Drawing for the job (mm, zero at the part's lowest x, y, z). A direction names the side the tool comes from. Round coordinates to 2 decimals unless told otherwise and drop trailing zeros. Loops run counter-clockwise (first coordinate to the right, second up) from the corner with the lowest first, then second, coordinate; pieces in that order, holes last. Notation, with made-up numbers: (-22, -31.5) -> (11, -31.5) arc R28 cw to (11, -1.5) -> close; hole circle Ø8 at (66, 71.5). An arc over 180 degrees is marked (long way). Put each result on its own line as item: value. Start each with the question number.
Item 1: Cut at C-C, the plane z = 2.5. List the corners of the cut face in (x, y).
Item 2: Drill centre lines: probe 1 along Y at (x, z) = (6, 2.5); probe 2 along Y at (x, z) = (8, 3.75); probe 3 along X at (y, z) = (4.25, 2.75). Where is each one in solid material? Low to high. Write a range as [from, to].
Item 3: Flat gauge pins, fed straight in: pin 1 Ø1.5 at (x, z) = (6, 2.5) entering from +Y; pin 2 Ø3.5 at (x, y) = (6.5, 7.5) entering from +Z; pin 3 Ø2 at (y, z) = (3.5, 1.5) entering from -X. Where does each tip first touch, or does it go through?
Item 4: Cut at B-B, the plane y = 6. List the corners of the cut face in (x, z), plus the area to 3 significant figures.
Item 5: Pull direction Y, two halves, no side cores. Call the marked faces 3, 4 and 5: +Y half, -Y half, draft (parallel to the pull), parting line (faces both ways), or undercut.
Item 6: Cut at A-A, the plane x = 6. List the corners of the cut face in (y, z).
Item 7: Tool access for the marked faces 1 and 2: list every direction of +Z, -Z, +X, -X, +Y, -Y with a clear straight run to the whole face (end or side of a thin tool).
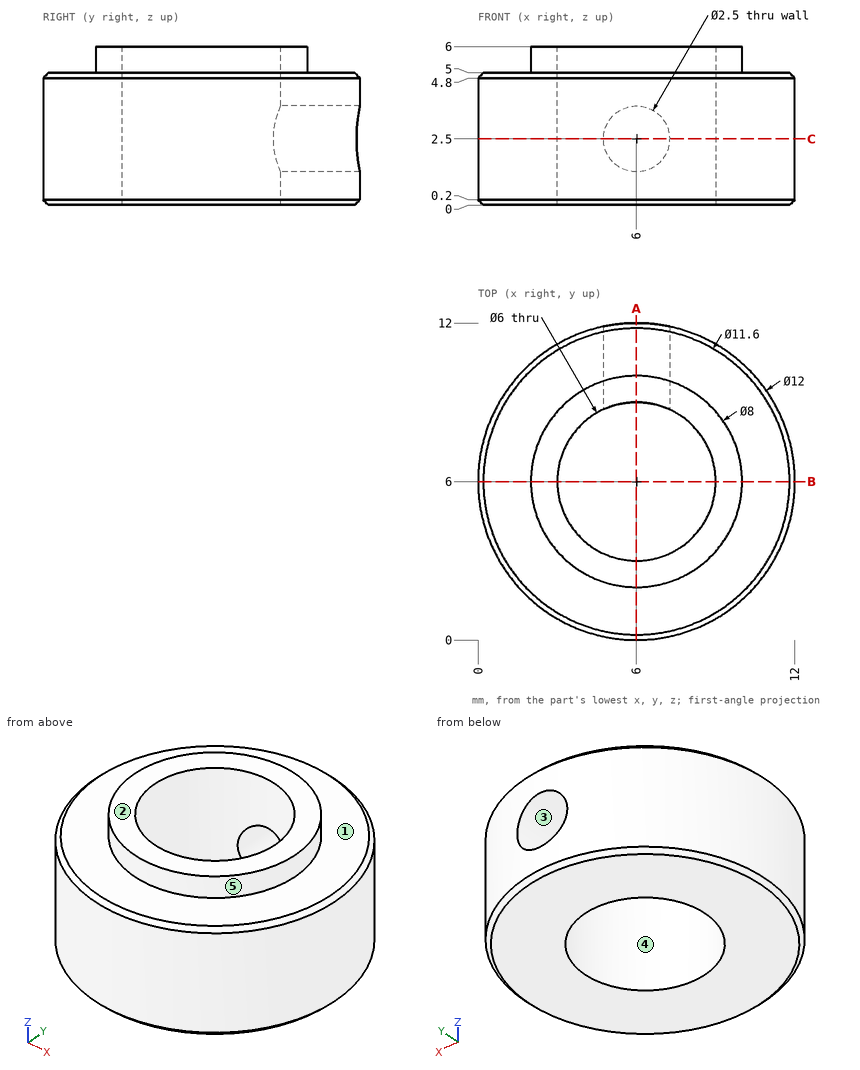
Reply:
1. outline: (4.75, 8.73) -> (4.75, 11.87) arc R6 ccw (long way) to (7.25, 11.87) -> (7.25, 8.73) arc R3 cw (long way) to start
2. probe 1: y = [0, 3]
2. probe 2: y = [0.34, 3.76], [8.24, 11.66]
2. probe 3: x = [0.26, 3.56], [8.44, 11.74]
3. pin 1: stops at y = 3.1
3. pin 2: stops at z = 6
3. pin 3: stops at x = 0.19
4. outline: (0, 0.2) -> (0.2, 0) -> (3, 0) -> (3, 6) -> (2, 6) -> (2, 5) -> (0.2, 5) -> (0, 4.8) -> close; (9, 0) -> (11.8, 0) -> (12, 0.2) -> (12, 4.8) -> (11.8, 5) -> (10, 5) -> (10, 6) -> (9, 6) -> close
4. area: 31.9 mm^2
5. face 3: draft
5. face 4: undercut
5. face 5: parting line
6. outline: (0, 0.2) -> (0.2, 0) -> (3, 0) -> (3, 6) -> (2, 6) -> (2, 5) -> (0.2, 5) -> (0, 4.8) -> close; (9, 0) -> (11.8, 0) -> (12, 0.2) -> (12, 1.25) -> (9, 1.25) -> close; (9, 3.75) -> (12, 3.75) -> (12, 4.8) -> (11.8, 5) -> (10, 5) -> (10, 6) -> (9, 6) -> close
7. face 1: +Z
7. face 2: +Z, +X, -X, +Y, -Y
